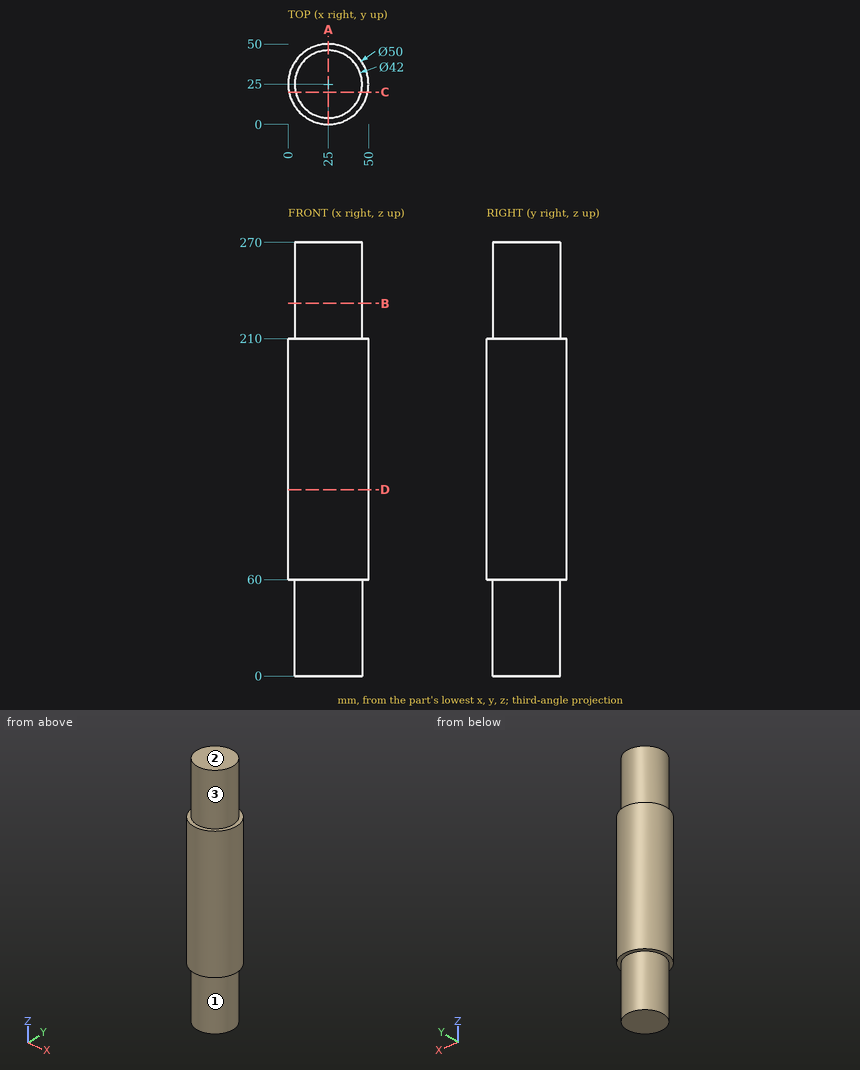
Could you check a few things on this drawing? It's one solid part, dimensions in mm from its lowest x, y, z. A direction names the side the tool comes from. Give positions to 0.01 mm unless a question says otherwise; leave off trailing zeros. Write each loop counter-clockwise with the first axis right and the second up, starting at its lowest first coordinate (ties: lowest second). Pieces come first, ordered by that corner, then holes. Notation, with made-up numbers: (-29, 48.5) -> (5, 48.5) arc R19 ccw to (5, 64.5) -> close; hole circle Ø1 at (47, -3). An arc over 180 degrees is marked (long way). Write item = value, one per line.
(1) I need wall thicknesses on probe 1 along Z at (x, y) = (33, 47); probe 2 along X at (y, z) = (25.5, 47); probe 3 along Y at (x, z) = (11.5, 182.5). Which ranges of each line are inside material? Lowest first, please. Write a range as from..to.
Worked out:
probe_1 = 60..210
probe_2 = 4.01..45.99
probe_3 = 3.96..46.04
(2) Suppose I cut it at C-C on y = 20. Write out the boundary of the cut face in (x, z), then the cut area to 3 significant figures.
Worked out:
outline = (0.51, 60) -> (4.6, 60) -> (4.6, 0) -> (45.4, 0) -> (45.4, 60) -> (49.49, 60) -> (49.49, 210) -> (45.4, 210) -> (45.4, 270) -> (4.6, 270) -> (4.6, 210) -> (0.51, 210) -> close
area = 12,200 mm^2
(3) I'm going to push flat-ended pins straight in: P1, Ø1.5, axis at x = 38.5, z = 131.5, coming from the -Y side; P2, Ø5, axis at y = 37, z = 236, coming from the -X side; P3, Ø1, axis at x = 42, z = 114, coming from the -Y side. Where does each tip first touch, or does it pass through?
Worked out:
P1 = 3.5
P2 = 6.27
P3 = 6.22
(4) Suppose I cut it at B-B on z = 232. Write out the boundary of the cut face in (x, y), then the cut area to 3 significant figures.
Worked out:
outline = circle Ø42 at (25, 25)
area = 1,390 mm^2
(5) Suppose I cut it at A-A on x = 25. Write out the boundary of the cut face in (y, z).
Worked out:
outline = (0, 60) -> (4, 60) -> (4, 0) -> (46, 0) -> (46, 60) -> (50, 60) -> (50, 210) -> (46, 210) -> (46, 270) -> (4, 270) -> (4, 210) -> (0, 210) -> close
(6) Suppose I cut it at D-D on z = 116. Write out the boundary of the cut face in (x, y), then the cut area to 3 significant figures.
Worked out:
outline = circle Ø50 at (25, 25)
area = 1,960 mm^2
(7) For the marked faces 1, 2 and 3, which set-ups out of +Z, -Z, +X, -X, +Y, -Y let a thin tool reach every point of the face, with its end or its side?
Worked out:
face_1 = -Z
face_2 = +Z, +X, -X, +Y, -Y
face_3 = +Z
